from build123d import *

# Parameters (mm, degrees)
BASE_PLATE_SKETCH_W     = 38.1
BASE_PLATE_SKETCH_H     = 63.5
BASE_PLATE_DEPTH        = 12.7
MOUNTING_HOLES_SKETCH_R = 6.35
MOUNTING_HOLES_DEPTH    = 112.622813528
INCLINED_LUG_REACH      = 102.603
LUG_BORE_REACH          = 102.603
LUG_BORE_SKETCH_R       = 7.62


with BuildPart() as part:
    # Base Plate Sketch → Base Plate (new body)
    with BuildSketch(Plane(origin=(0, 0, 0), x_dir=(1, 0, 0), z_dir=(0, 1, 0))):
        with BuildLine():
            Line((31.75, 12.7), (-31.75, 12.7))
            ThreePointArc((-31.75, 12.7), (-44.45, 0), (-31.75, -12.7))
            Line((-31.75, -12.7), (31.75, -12.7))
            ThreePointArc((31.75, -12.7), (44.45, 0), (31.75, 12.7))
        make_face()
        with Locations((0, -44.45)):
            Rectangle(BASE_PLATE_SKETCH_W, BASE_PLATE_SKETCH_H)
        with BuildLine():
            Line((31.75, -76.2), (-31.75, -76.2))
            ThreePointArc((-31.75, -76.2), (-44.45, -88.9), (-31.75, -101.6))
            Line((-31.75, -101.6), (31.75, -101.6))
            ThreePointArc((31.75, -101.6), (44.45, -88.9), (31.75, -76.2))
        make_face()
    extrude(amount=BASE_PLATE_DEPTH)

    # Mounting Holes Sketch → Mounting Holes (cut, through all)
    with BuildSketch(Plane(origin=(0, 12.7, 0), x_dir=(1, 0, 0), z_dir=(0, 1, 0))):
        with Locations(Location((-31.75, 0, 0), (0, 0, 270))):
            Circle(MOUNTING_HOLES_SKETCH_R)
        with Locations(Location((31.75, 0, 0), (0, 0, 270))):
            Circle(MOUNTING_HOLES_SKETCH_R)
        with Locations(Location((-31.75, -88.9, 0), (0, 0, 270))):
            Circle(MOUNTING_HOLES_SKETCH_R)
        with Locations(Location((31.75, -88.9, 0), (0, 0, 270))):
            Circle(MOUNTING_HOLES_SKETCH_R)
        with BuildLine():
            Line((-6.35, 0), (-6.35, 12.7))
            Line((-6.35, 12.7), (6.35, 12.7))
            Line((6.35, 12.7), (6.35, 0))
            ThreePointArc((6.35, 0), (0, -6.35), (-6.35, 0))
        make_face()
    extrude(amount=-MOUNTING_HOLES_DEPTH, mode=Mode.SUBTRACT)

    # Inclined Lug Sketch → Inclined Lug (add, up to next)
    with BuildSketch(Plane(origin=(0, 57.15, 57.15), x_dir=(-1, 0, 0), z_dir=(0, 0.7071067811865488, 0.7071067811865464)), mode=Mode.PRIVATE) as inclined_lug_sk1:
        with BuildLine():
            Line((-19.05, 62.861792847), (19.05, 62.861792847))
            Line((19.05, 62.861792847), (19.05, 27.809792847))
            ThreePointArc((19.05, 27.809792847), (0, 8.759792847), (-19.05, 27.809792847))
            Line((-19.05, 27.809792847), (-19.05, 62.861792847))
        make_face()
    inclined_lug_tool1 = extrude(inclined_lug_sk1.sketch, amount=-INCLINED_LUG_REACH, mode=Mode.PRIVATE) - part.part
    add(inclined_lug_tool1.solids().sort_by_distance((0, 30.51036, 83.78964))[0])

    # Lug Bore: up to this plane
    lug_bore_end = Plane(origin=(0, 0, 0), z_dir=(0, 1, 0))
    # Lug Bore Sketch → Lug Bore (cut, up to the surface)
    with BuildSketch(Plane(origin=(0, 57.15, 57.15), x_dir=(1, 0, 0), z_dir=(0, 0.7071067811865487, 0.7071067811865465)), mode=Mode.PRIVATE) as lug_bore_sk1:
        with Locations(Location((0, -27.809792847, 0), (0, 0, 270))):
            Circle(LUG_BORE_SKETCH_R)
    lug_bore_tool1 = split(extrude(lug_bore_sk1.sketch, amount=-LUG_BORE_REACH, mode=Mode.PRIVATE), bisect_by=lug_bore_end, keep=Keep.BOTH, mode=Mode.PRIVATE)
    add(lug_bore_tool1.solids().sort_by_distance((0, 37.485507, 76.814493))[0], mode=Mode.SUBTRACT)


solid = part.part
The listing builds one solid part. Answer for the finished solid, in the listing's coordinates (mm). A direction names the side the tool comes from. Coordinates: 2 decimals unless noted, no trailing zeros. Order: outer loops, then holes, each group sorted by start corner. A loop starts at its lowest first (then second) coordinate and runs counter-clockwise, first axis right, second up. Notation, with made-up numbers: (59, -31) -> (94, -31) arc R26 cw to (94, 4) -> close; hole circle Ø9 at (-18.75, -8.75). An arc over 180 degrees is marked (long way). Answer in a Markdown table with one row per item. Add a question column.
Item 1: Which of the six approach directions +Z, -Z, +X, -X, +Y, -Y give full straight-line access (tool end or side, diameter ignored) to faces 4 (the face through (-25, 6, 12.7)), 5 (the face through (26, 12.7, 92)), 6 (the face through (19.05, 14, 58))?
Item 2: Find the intervals of material crossed by L1, parallel to X at y = 5, z = 88; L2, parallel to X at y = 5.5, z = 35; L3, parallel to Y at x = 40, z = 84, in increasing order. Write a range as from..to.
Item 3: Find section D-D (x = 0). Write down the section's boundary in (y, z).
Item 4: Determine the mould class of faces 1 (the face through (0.14, 6.44, 6.35)), 2 (the face through (32.029, 6.439, 82.556)), 3 (the face through (0, 6, 101.6)) for opening direction Z: +Z half, -Z half, draft (parallel to the pull), parting line (faces both ways), or undercut.
Item 5: Find section C-C (z = -4). Write down the section's boundary in (x, y), then the cut area to 3 significant figures.
Item 6: Each of these flat-tipped pins is pushed along its axis until it touches: P1, Ø10, axis at y = 4.5, z = -9, coming from the +X side; P2, Ø10, axis at y = 3, z = -9, coming from the -X side; P3, Ø10, axis at y = 19, z = 54, coming from the -X side. Where does it stop, or does it pass through?
Item 7: Find section B-B (z = 88.9). Write down the section's boundary in (x, y).
Item 8: Find section A-A (x = 24). Write down the section's boundary in (y, z), then the cut area to 3 significant figures.
Result set:
| question | item | result |
|---|---|---|
| 1 | face 4 | -X, +Y, -Y |
| 1 | face 5 | +Z, -Z, +X, +Y |
| 1 | face 6 | +X, +Y |
| 2 | L1 | x = -44.42..-38.04, -25.46..25.46, 38.04..44.42 |
| 2 | L2 | x = -19.05..-3.12, 3.12..19.05 |
| 2 | L3 | y = 0..12.7 |
| 3 | outline | (0, 6.35) -> (12.7, 6.35) -> (12.7, 25.09) -> (50.96, 63.34) -> (42.87, 71.43) -> (0, 28.55) -> close; (0, 50.11) -> (32.1, 82.2) -> (12.7, 101.6) -> (0, 101.6) -> close |
| 4 | face 1 | -Z half |
| 4 | face 2 | undercut |
| 4 | face 3 | +Z half |
| 5 | outline | (-43.8, 0) -> (-36.68, 0) -> (-36.68, 12.7) -> (-43.8, 12.7) -> close; (-26.82, 0) -> (-6.35, 0) -> (-6.35, 12.7) -> (-26.82, 12.7) -> close; (6.35, 0) -> (26.82, 0) -> (26.82, 12.7) -> (6.35, 12.7) -> close; (36.68, 0) -> (43.8, 0) -> (43.8, 12.7) -> (36.68, 12.7) -> close |
| 5 | area | 701 mm² |
| 6 | P1 | stops at x = 43.8 |
| 6 | P2 | stops at x = -43.8 |
| 6 | P3 | stops at x = -19.05 |
| 7 | outline | (-44.45, 0) -> (-38.1, 0) -> (-38.1, 12.7) -> (-44.45, 12.7) -> close; (-25.4, 0) -> (25.4, 0) -> (25.4, 12.7) -> (19.05, 12.7) -> (19.05, 25.4) -> (-19.05, 25.4) -> (-19.05, 12.7) -> (-25.4, 12.7) -> close; (38.1, 0) -> (44.45, 0) -> (44.45, 12.7) -> (38.1, 12.7) -> close |
| 8 | outline | (0, -12.7) -> (12.7, -12.7) -> (12.7, 12.7) -> (0, 12.7) -> close; (0, 76.2) -> (12.7, 76.2) -> (12.7, 101.6) -> (0, 101.6) -> close |
| 8 | area | 645 mm² |
